from build123d import *

# Parameters (mm, degrees)
SKETCH2_W              = 80
SKETCH2_H              = 126
BOSS_EXTRUDE1_DEPTH    = 63
M36_TAPPED_HOLE1_D     = 32
M36_TAPPED_HOLE1_DEPTH = 80
M36_TAPPED_HOLE1_TIP   = 9.613769904


with BuildPart() as part:
    # Sketch2 → Boss-Extrude1 (new, symmetric)
    with BuildSketch(Plane(origin=(0, 0, 0), x_dir=(1, 0, 0), z_dir=(0, 1, 0))):
        Rectangle(SKETCH2_W, SKETCH2_H)
    extrude(amount=BOSS_EXTRUDE1_DEPTH, both=True)

    # M36 Tapped Hole1
    with Locations(Plane(origin=(0, 63, 0), x_dir=(1, 0, 0), z_dir=(0, 1, 0))):
        with Locations((0, 34), (0, -34)):
            Hole(M36_TAPPED_HOLE1_D / 2, depth=M36_TAPPED_HOLE1_DEPTH)
            with Locations((0, 0, -(M36_TAPPED_HOLE1_DEPTH + M36_TAPPED_HOLE1_TIP / 2))):  # 118° drill point
                Cone(0, M36_TAPPED_HOLE1_D / 2, M36_TAPPED_HOLE1_TIP, mode=Mode.SUBTRACT)


solid = part.part
Check sheet for the modelled part. Datum: model origin and axes. Units: mm. A direction names the side the tool comes from. Give positions to 0.01 mm unless a question says otherwise; leave off trailing zeros. Order: outer loops, then holes, each group sorted by start corner. A loop starts at its lowest first (then second) coordinate and runs counter-clockwise, first axis right, second up. Notation, with made-up numbers: (-18, 16.25) - (24, 16.25) arc R22 cw to (24, 45.25) - close; hole circle Ø9 at (45, 1). An arc over 180 degrees is marked (long way). Answer as CSV lines item,"result".
1. Scan lines: probe 1 along Z at (x, y) = (0, 46); probe 2 along Z at (x, y) = (6, 58); probe 3 along X at (y, z) = (-5, 23.5). Record each from-to range of solid material in increasing order. Write a range as from..to.
Result sheet:
probe 1,"-63..-50, -18..18, 50..63"
probe 2,"-63..-48.83, -19.17..19.17, 48.83..63"
probe 3,"-40..-12.07, 12.07..40"
2. Mould release check, pull along Z, two halves, no side actions. Record for faces 3 (the face through (1.28, -24.94, 36.47)), 4 (the face through (-40, 1, 1)), 5 (the face through (-1, 1, 63)): released by +Z, released by -Z, zero draft, split by the parting line, or undercut.
Result sheet:
face 3,"undercut"
face 4,"zero draft"
face 5,"released by +Z"
3. Tool access check on faces 1 (the face through (-1, -63, -1)), 2 (the face through (3.47, 22.44, -18.38)). Record the directions out of +Z, -Z, +X, -X, +Y, -Y that give a thin tool (end or side, any length) a straight path to the whole face; none if there is none.
Result sheet:
face 1,"+Z, -Z, +X, -X, -Y"
face 2,"+Y"
4. Section check B-B (y = -20). Record the boundary of the cut face in (x, z), then the cut area to 3 significant figures.
Result sheet:
outline,"(-40, -63) - (40, -63) - (40, 63) - (-40, 63) - close; hole circle Ø22.01 at (0, -34); hole circle Ø22.01 at (0, 34)"
area,"9,320 mm²"
5. Section check A-A (y = -1). Record the boundary of the cut face in (x, z).
Result sheet:
outline,"(-40, -63) - (40, -63) - (40, 63) - (-40, 63) - close; hole circle Ø32 at (0, -34); hole circle Ø32 at (0, 34)"
